from build123d import *

# Parameters (mm, degrees)
BASE_PLATE_SKETCH_W      = 127
BASE_PLATE_SKETCH_H      = 127
BASE_PLATE_DEPTH         = 12.7
UPRIGHT_WALL_SKETCH_W    = 127
UPRIGHT_WALL_SKETCH_H    = 12.7
UPRIGHT_WALL_DEPTH       = 127
GUSSET_1_DEPTH           = 12.7
GUSSET_2_DEPTH           = 12.7
MOUNTING_HOLE_1_SKETCH_R = 12.7
MOUNTING_HOLE_1_DEPTH    = 12.7
MOUNTING_HOLE_2_SKETCH_R = 12.7
MOUNTING_HOLE_2_DEPTH    = 12.7
MOUNTING_HOLE_3_SKETCH_R = 12.7
MOUNTING_HOLE_3_DEPTH    = 12.7
MOUNTING_HOLE_4_SKETCH_R = 12.7
MOUNTING_HOLE_4_DEPTH    = 12.7


with BuildPart() as part:
    # Base Plate Sketch → Base Plate (new body)
    with BuildSketch(Plane.XY):
        with Locations((63.5, 63.5)):
            Rectangle(BASE_PLATE_SKETCH_W, BASE_PLATE_SKETCH_H)
    extrude(amount=BASE_PLATE_DEPTH)

    # Upright Wall Sketch → Upright Wall (add)
    with BuildSketch(Plane.XY.offset(12.7)):
        with Locations((63.5, 120.65)):
            Rectangle(UPRIGHT_WALL_SKETCH_W, UPRIGHT_WALL_SKETCH_H)
    extrude(amount=UPRIGHT_WALL_DEPTH)

    # Gusset 1 Sketch → Gusset 1 (add)
    with BuildSketch(Plane.ZY):
        Polygon((12.7, 0), (139.7, 114.3), (12.7, 114.3), align=None)
    extrude(amount=-GUSSET_1_DEPTH)

    # Gusset 2 Sketch → Gusset 2 (add)
    with BuildSketch(Plane(origin=(127, 0, 0), x_dir=(0, 0, -1), z_dir=(1, 0, 0))):
        Polygon((-12.7, 0), (-12.7, 114.3), (-139.7, 114.3), align=None)
    extrude(amount=-GUSSET_2_DEPTH)

    # Mounting Hole 1 Sketch → Mounting Hole 1 (cut)
    with BuildSketch(Plane.XZ.offset(-114.3)):
        with Locations(Location((38.1, 101.6, 0), (0, 0, 270))):
            Circle(MOUNTING_HOLE_1_SKETCH_R)
    extrude(amount=-MOUNTING_HOLE_1_DEPTH, mode=Mode.SUBTRACT)

    # Mounting Hole 2 Sketch → Mounting Hole 2 (cut)
    with BuildSketch(Plane.XZ.offset(-114.3)):
        with Locations(Location((88.9, 101.6, 0), (0, 0, 270))):
            Circle(MOUNTING_HOLE_2_SKETCH_R)
    extrude(amount=-MOUNTING_HOLE_2_DEPTH, mode=Mode.SUBTRACT)

    # Mounting Hole 3 Sketch → Mounting Hole 3 (cut)
    with BuildSketch(Plane.XY.offset(12.7)):
        with Locations((37.774003387, 25.4)):
            Circle(MOUNTING_HOLE_3_SKETCH_R)
    extrude(amount=-MOUNTING_HOLE_3_DEPTH, mode=Mode.SUBTRACT)

    # Mounting Hole 4 Sketch → Mounting Hole 4 (cut)
    with BuildSketch(Plane.XY.offset(12.7)):
        with Locations((91.0635678, 25.4)):
            Circle(MOUNTING_HOLE_4_SKETCH_R)
    extrude(amount=-MOUNTING_HOLE_4_DEPTH, mode=Mode.SUBTRACT)


solid = part.part
The model under review builds one solid part; all positions refer to its coordinate system, in mm. A direction names the side the tool comes from. Give positions to 0.01 mm unless a question says otherwise; leave off trailing zeros. Order: outer loops, then holes, each group sorted by start corner. A loop starts at its lowest first (then second) coordinate and runs counter-clockwise, first axis right, second up. Notation, with made-up numbers: M -9.5,1 L 18.5,1 A18 ccw 18.5,25 Z; hole C -39,31 d9. An arc over 180 degrees is marked long. Use one line per item in the form item = value. Start each with the question number.
Item 1: To check wall thickness, follow line 1 along X through (y, z) = (99, 118); line 2 along X through (y, z) = (123, 101.6); line 3 along X through (y, z) = (14, 10). State the ranges of each line that lie inside material, in increasing order. Write a range as from..to.
Item 2: We need section D-D on y = 30. Give the boundary of the cut face in (x, z).
Item 3: The part is to be moulded in two halves that separate along Z. For faces 1 (the flat face through (63, 0, 6)), 2 (the cylindrical face through (92.715, 120.561, 89.486)), 3 (the flat face through (63, 64, 0)), say which applies: pulls with the +Z half, pulls with the -Z half, needs draft (parallel to the pull), parting line crosses it, or undercut.
Item 4: We need section C-C on x = 91. Give the boundary of the cut face in (y, z).
Item 5: We need section A-A on z = 101.6. Give the boundary of the cut face in (x, y), plus the area to 3 significant figures.
Item 6: For faces 4 (the flat face through (120.74, 57.95, 77.09)), 5 (the flat face through (63, 58, 12.7)), list the 3-axis set-ups (+Z, -Z, +X, -X, +Y, -Y) from which the entire face can be reached by the end or side of a thin tool; tool diameter is ignored.
Item 7: Insertion check: pin 1 Ø8 at (x, y) = (38.5, 99.5) entering from -Z; pin 2 Ø4 at (x, z) = (94.5, 66) entering from -Y; pin 3 Ø3 at (x, y) = (84, 97.5) entering from +Z. Each pin has a flat end and moves straight along its axis. Give the tip position at first contact, or say it passes through.
Item 8: We need section B-B on z = 30. Give the boundary of the cut face in (x, y), plus the area to 3 significant figures.
Completed:
q1.line_1 = 0..12.7, 114.3..127
q1.line_2 = 0..25.4, 50.8..76.2, 101.6..127
q1.line_3 = 0..32.18, 43.37..85.47, 96.66..127
q2.outline = M 0,0 L 25.94,0 L 25.94,12.7 L 12.7,12.7 L 12.7,46.03 L 0,46.03 Z; M 49.61,0 L 79.23,0 L 79.23,12.7 L 49.61,12.7 Z; M 102.9,0 L 127,0 L 127,46.03 L 114.3,46.03 L 114.3,12.7 L 102.9,12.7 Z
q3.face_1 = needs draft
q3.face_2 = undercut
q3.face_3 = pulls with the -Z half
q4.outline = M 0,0 L 12.7,0 L 12.7,12.7 L 0,12.7 Z; M 38.1,0 L 127,0 L 127,89.07 L 114.3,89.07 L 114.3,12.7 L 38.1,12.7 Z; M 114.3,114.13 L 127,114.13 L 127,139.7 L 114.3,139.7 Z
q5.outline = M 0,80.01 L 12.7,80.01 L 12.7,114.3 L 25.4,114.3 L 25.4,127 L 0,127 Z; M 50.8,114.3 L 76.2,114.3 L 76.2,127 L 50.8,127 Z; M 101.6,114.3 L 114.3,114.3 L 114.3,80.01 L 127,80.01 L 127,127 L 101.6,127 Z
q5.area = 1,840 mm²
q6.face_4 = +Z, +X, -X, -Y
q6.face_5 = +Z, -Y
q7.pin_1 = 0
q7.pin_2 = 114.3
q7.pin_3 = 12.7
q8.outline = M 0,15.57 L 12.7,15.57 L 12.7,114.3 L 114.3,114.3 L 114.3,15.57 L 127,15.57 L 127,127 L 0,127 Z
q8.area = 4,120 mm²
